Could you check a few things on this model? Use its own coordinates, in mm. A direction names the side the tool comes from. Coordinates: 2 decimals unless noted, no trailing zeros. Loops run counter-clockwise (first coordinate to the right, second up) from the corner with the lowest first, then second, coordinate; pieces in that order, holes last. Notation, with made-up numbers: M -30,21.25 L -4,21.25 A23 ccw -4,40.25 Z; hole C -27,7 d3. An arc over 180 degrees is marked long. Return JSON: item names as keys, results as strings. Group by question number.
from build123d import *

# Parameters (mm, degrees)
SKETCH1_R           = 12.5
SKETCH1_R_2         = 6.5
BOSS_EXTRUDE1_DEPTH = 4


with BuildPart() as part:
    # Sketch1 → Boss-Extrude1 (new, symmetric)
    with BuildSketch(Plane.XY):
        with BuildLine():
            Line((50, 0), (-50, 0))
            Line((-50, 0), (-45.028143867, 114.700831063))
            ThreePointArc((-45.028143867, 114.700831063), (-45.989821567, 123.642613906), (-49.558557115, 131.897577927))
            Line((-49.558557115, 131.897577927), (-87.251556293, 192.218986015))
            ThreePointArc((-87.251556293, 192.218986015), (-85.713994314, 205.713994314), (-72.218986015, 207.251556293))
            Line((-72.218986015, 207.251556293), (-21.196770569, 175.369337595))
            ThreePointArc((-21.196770569, 175.369337595), (-11.025494233, 170.840793604), (0, 169.291261441))
            ThreePointArc((0, 169.291261441), (11.025494233, 170.840793604), (21.196770569, 175.369337595))
            Line((21.196770569, 175.369337595), (72.218986015, 207.251556293))
            ThreePointArc((72.218986015, 207.251556293), (85.713994314, 205.713994314), (87.251556293, 192.218986015))
            Line((87.251556293, 192.218986015), (49.558557115, 131.897577927))
            ThreePointArc((49.558557115, 131.897577927), (45.989821567, 123.642613906), (45.028143867, 114.700831063))
            Line((45.028143867, 114.700831063), (50, 0))
        make_face()
        with Locations((0, 120)):
            Circle(SKETCH1_R, mode=Mode.SUBTRACT)
        with Locations((78, 198)):
            Circle(SKETCH1_R_2, mode=Mode.SUBTRACT)
        with Locations(Location((-78, 198, 0), (0, 0, 180))):
            Circle(SKETCH1_R_2, mode=Mode.SUBTRACT)
    extrude(amount=BOSS_EXTRUDE1_DEPTH, both=True)


solid = part.part
(1) Imagine slicing it at D-D, the plane y = 198. Write out the boundary of the cut face in (x, z).
(2) Will these pins go through, and if not, where does the flat tip stop? P1, Ø1.5, axis at y = 151, z = -0.5, coming from the -X side; P2, Ø1, axis at x = 11.5, z = -3, coming from the +Y side; P3, Ø2, axis at y = 159.5, z = -1.5, coming from the +X side.
(3) We'd pull the mould along X, two halves only. Please class faces 1 (the face through (-47.065, 191.534, 0.056)), 2 (the face through (-47.55, 56.55, 0.06)), 3 (the face through (46.02, 123.76, 0.06)): +X half, -X half, draft (parallel to the pull), parting line (faces both ways), or undercut.
(4) For faces 4 (the face through (47.48, 58.15, 0.06)), 5 (the face through (68.67, 162.48, 0.06)), 6 (the face through (-45.958, 123.52, 0.056)), 7 (the face through (46.351, 191.087, 0.056)), 8 (the face through (-85.858, 205.568, 0.056)), which set-ups out of +Z, -Z, +X, -X, +Y, -Y let a thin tool reach every point of the face, with its end or its side?
(5) If I drill on L1, parallel to Y at x = 0, z = -2; L2, parallel to X at y = 108.5, z = -2.5; L3, parallel to Y at x = -78, z = -1.5, over which ranges is the centre line in solid material (lowest first)? Write a range as [from, to].
(6) Imagine slicing it at B-B, the plane x = 0. Write out the boundary of the cut face in (y, z).
(7) Imagine slicing it at A-A, the plane z = 1.75. Write out the boundary of the cut face in (x, y).
(8) Imagine slicing it at C-C, the plane y = 129. Write out the boundary of the cut face in (x, z), then the cut area to 3 significant figures.
Checks:
{
 "1": {"outline": "M -88.91,-4 L -84.5,-4 L -84.5,4 L -88.91,4 Z; M -71.5,-4 L -57.41,-4 L -57.41,4 L -71.5,4 Z; M 57.41,-4 L 71.5,-4 L 71.5,4 L 57.41,4 Z; M 84.5,-4 L 88.91,-4 L 88.91,4 L 84.5,4 Z"},
 "2": {"P1": "x = -61.96", "P2": "y = 171.13", "P3": "x = 67.43"},
 "3": {"face 1": "undercut", "face 2": "-X half", "face 3": "+X half"},
 "4": {"face 4": "+Z, -Z, +X", "face 5": "+Z, -Z, +X, -Y", "face 6": "+Z, -Z, -X", "face 7": "+Z, -Z, +Y", "face 8": "+Z, -Z"},
 "5": {"L1": "[0, 107.5], [132.5, 169.29]", "L2": "[-45.3, -4.9], [4.9, 45.3]", "L3": "[177.41, 191.5], [204.5, 208.91]"},
 "6": {"outline": "M 0,-4 L 107.5,-4 L 107.5,4 L 0,4 Z; M 132.5,-4 L 169.29,-4 L 169.29,4 L 132.5,4 Z"},
 "7": {"outline": "M -87.25,192.22 L -49.56,131.9 A30 cw -45.03,114.7 L -50,0 L 50,0 L 45.03,114.7 A30 cw 49.56,131.9 L 87.25,192.22 A10.91 ccw 72.22,207.25 L 21.2,175.37 A40 cw -21.2,175.37 L -72.22,207.25 A10.91 ccw Z; hole C -78,198 d13; hole C 0,120 d25; hole C 78,198 d13"},
 "8": {"outline": "M -47.96,-4 L -8.67,-4 L -8.67,4 L -47.96,4 Z; M 8.67,-4 L 47.96,-4 L 47.96,4 L 8.67,4 Z", "area": "629 mm²"}
}
